Input: part model. Units: mm. Frame: model coordinates. A direction names the side the tool comes from. Give positions to 0.01 mm unless a question says otherwise; leave off trailing zeros. Loops run counter-clockwise (first coordinate to the right, second up) from the corner with the lowest first, then second, coordinate; pieces in that order, holes last. Notation, with made-up numbers: M 20.25,55 L 71.25,55 A11 ccw 71.25,74 Z; hole C -10.75,68 d10. An arc over 180 degrees is marked long. Answer as a JSON object with one key per item and string values. Group by question number.
1) Section query A-A on x = 0. Return loops of the section in (y, z).
2) Ray query, L1, parallel to Z at x = 0, y = 6.5; L2, parallel to Y at x = 4.25, z = 4; L3, parallel to Z at x = 2.75, y = 12.5. Return the intervals inside material, ascending.
3) Access query for faces 5 (the flat face through (4, 14, -4)), 6 (the flat face through (0, 7, 6)), 7 (the cylindrical face through (1.802, 14.986, 5.723)). Directions: +Z, -Z, +X, -X, +Y, -Y. A direction counts if a zero-diameter tool reaches every point of the face in a straight line with its end or side. Return the directions, or none.
4) Section query D-D on x = 5.5. Return loops of the section in (y, z), plus the area to 3 significant figures.
5) Section query B-B on y = 13. Return loops of the section in (x, z).
6) Draft query along Y for faces 1 (the flat face through (-1, 16, 3)), 2 (the cylindrical face through (-4.88, 13.75, -1.08)), 3 (the flat face through (1, 0, -3)), 4 (the flat face through (0, 7, -6)). Return one class per face: +Y half, -Y half, draft (parallel to the pull), parting line (faces both ways), or undercut.
7) First-contact query: P1, Ø4, axis at y = 5.5, z = -3, coming from the +X side; P2, Ø5, axis at y = 9.5, z = -5, coming from the -X side; P3, Ø3, axis at y = 7.5, z = -4.5, coming from the -X side. Flat tips, straight axial feed; report the tip coordinate or a pass-through.
8) Section query C-C on z = -2. Return loops of the section in (x, y).
from build123d import *

# Parameters (mm, degrees)
BOSS_EXTRUDE1_DEPTH = 13.5
HOLE1_D             = 6


with BuildPart() as part:
    # Sketch1 → Boss-Extrude1 (new body)
    with BuildSketch(Plane(origin=(0, 0, 0), x_dir=(1, 0, 0), z_dir=(0, 1, 0))):
        Polygon((-6.92820323, 0), (-3.464101615, -6), (3.464101615, -6), (6.92820323, 0), (3.464101615, 6), (-3.464101615, 6), align=None)
    extrude(amount=BOSS_EXTRUDE1_DEPTH)

    # Sketch2 → Revolve1 (revolve)
    with BuildSketch(Plane.XY, mode=Mode.PRIVATE) as revolve1_sk:
        Polygon((0, 16), (6, 16), (6, 14), (5, 14), (5, 13.5), (0, 13.5), align=None)
    revolve(revolve1_sk.sketch.rotate(Axis((0, 13.5, 0), (0, 1, 0)), 270), axis=Axis((0, 13.5, 0), (0, 1, 0)))

    # Hole1 (through all)
    with Locations(Plane(origin=(0, 0, 0), x_dir=(-1, 0, 0), z_dir=(0, -1, 0))):
        with Locations((0, 0)):
            Hole(HOLE1_D / 2)


solid = part.part
Output:
{
 "1": {"outline": "M 0,-6 L 13.5,-6 L 13.5,-5 L 14,-5 L 14,-6 L 16,-6 L 16,-3 L 0,-3 Z; M 0,3 L 16,3 L 16,6 L 14,6 L 14,5 L 13.5,5 L 13.5,6 L 0,6 Z"},
 "2": {"L1": "z = -6 to -3, 3 to 6", "L2": "y = 0 to 13.5, 14 to 16", "L3": "z = -6 to -1.2, 1.2 to 6"},
 "3": {"face 5": "none", "face 6": "+Z, +X, -X, +Y, -Y", "face 7": "+Y"},
 "4": {"outline": "M 0,-2.47 L 13.5,-2.47 L 13.5,2.47 L 0,2.47 Z; M 14,-2.4 L 16,-2.4 L 16,2.4 L 14,2.4 Z", "area": "76.4 mm^2"},
 "5": {"outline": "M -6.93,0 L -3.46,-6 L 3.46,-6 L 6.93,0 L 3.46,6 L -3.46,6 Z; hole C 0,0 d6"},
 "6": {"face 1": "+Y half", "face 2": "undercut", "face 3": "-Y half", "face 4": "draft"},
 "7": {"P1": "stops at x = 6.35", "P2": "stops at x = -5.48", "P3": "stops at x = -5.2"},
 "8": {"outline": "M -5.77,0 L -2.24,0 L -2.24,16 L -5.66,16 L -5.66,14 L -4.58,14 L -4.58,13.5 L -5.77,13.5 Z; M 2.24,0 L 5.77,0 L 5.77,13.5 L 4.58,13.5 L 4.58,14 L 5.66,14 L 5.66,16 L 2.24,16 Z"}
}
